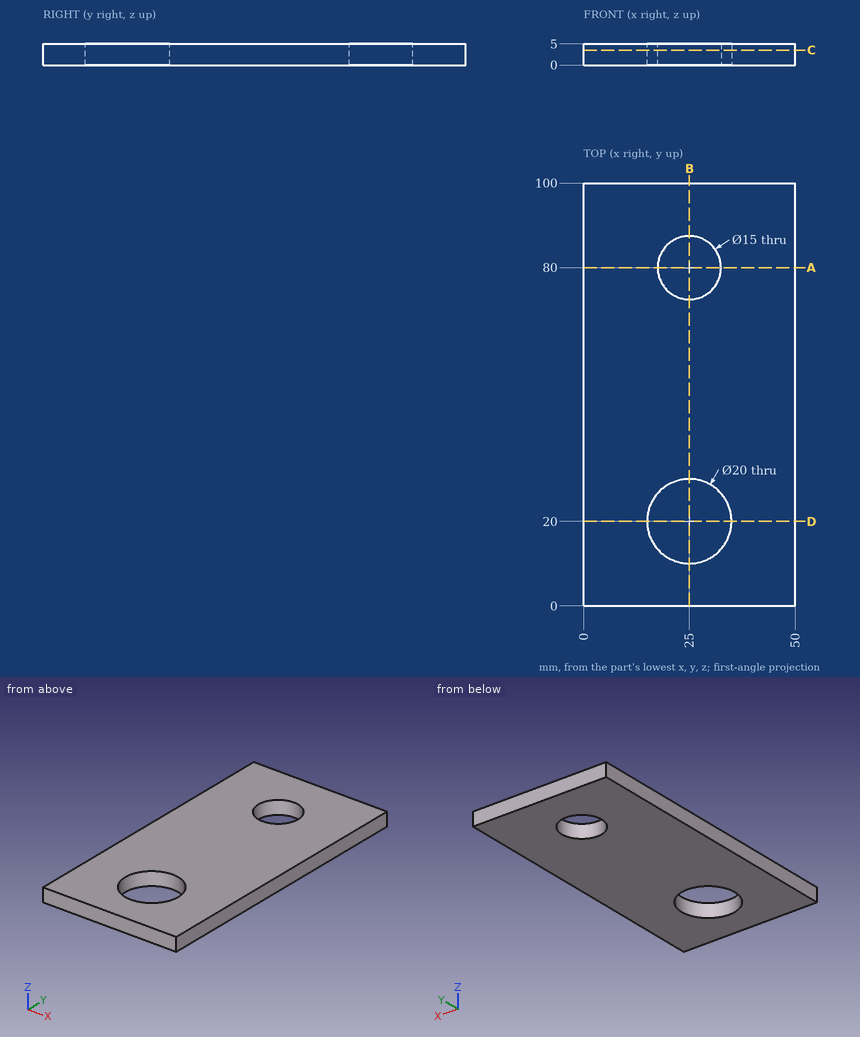
Part print with two shaded views. Sizes in mm from the minimum x, y, z corner. Round coordinates to 2 decimals unless told otherwise and drop trailing zeros. Loops run counter-clockwise (first coordinate to the right, second up) from the corner with the lowest first, then second, coordinate; pieces in that order, holes last. Notation, with made-up numbers: M 62.5,-13 L 80.5,-13 A19 cw 80.5,2 Z; hole C 42,65.5 d9. An arc over 180 degrees is marked long. Return JSON: item names as keys, results as strings. Group by question number.
(1) Saw through at D-D, the plane y = 20. List the corners of the cut face in (x, z).
(2) Saw through at A-A, the plane y = 80. List the corners of the cut face in (x, z).
(3) Wall check: probe 1 along Y at (x, z) = (25, 3.45); probe 2 along Y at (x, z) = (29.5, 2); probe 3 along X at (y, z) = (77, 4.7). Give the ranges that are in metal, low to high. Write a range as [from, to].
(4) Saw through at C-C, the plane z = 3.55. List the corners of the cut face in (x, y).
(5) Saw through at B-B, the plane x = 25. List the corners of the cut face in (y, z), and give its area (3 significant figures).
Answer list:
{
 "1": {"outline": "M 0,0 L 15,0 L 15,5 L 0,5 Z; M 35,0 L 50,0 L 50,5 L 35,5 Z"},
 "2": {"outline": "M 0,0 L 17.5,0 L 17.5,5 L 0,5 Z; M 32.5,0 L 50,0 L 50,5 L 32.5,5 Z"},
 "3": {"probe 1": "[0, 10], [30, 72.5], [87.5, 100]", "probe 2": "[0, 11.07], [28.93, 74], [86, 100]", "probe 3": "[0, 18.13], [31.87, 50]"},
 "4": {"outline": "M 0,0 L 50,0 L 50,100 L 0,100 Z; hole C 25,20 d20; hole C 25,80 d15"},
 "5": {"outline": "M 0,0 L 10,0 L 10,5 L 0,5 Z; M 30,0 L 72.5,0 L 72.5,5 L 30,5 Z; M 87.5,0 L 100,0 L 100,5 L 87.5,5 Z", "area": "325 mm2"}
}
